```python
from build123d import *

# Parameters (mm, degrees)
L_BRACKET_BODY_DEPTH           = 100
MOUNTING_HOLES_SKETCH_R        = 7
MOUNTING_HOLES_2X_14_DEPTH     = 100
TRUNNION_SKETCH_R              = 20
TRUNNION_40_DEPTH              = 100
TRUNNION_START                 = 5
TRUNNION_END_BOSS_A_SKETCH_R   = 20
TRUNNION_END_BOSS_A_40X5_DEPTH = 5
TRUNNION_END_BOSS_B_SKETCH_R   = 20
TRUNNION_END_BOSS_B_40X5_DEPTH = 5
TRUNNION_BORE_SKETCH_R         = 10
TRUNNION_BORE_20_DEPTH         = 110


with BuildPart() as part:
    # L Bracket Profile Sketch → L Bracket Body (new body)
    with BuildSketch(Plane.XY):
        Polygon((0, 0), (125, 0), (125, 42.5), (16, 42.5), (16, 85), (0, 85), align=None)
    extrude(amount=-L_BRACKET_BODY_DEPTH)

    # Mounting Holes Sketch → Mounting Holes 2xØ14 (cut)
    with BuildSketch(Plane(origin=(16, 0, 0), x_dir=(0, 0, -1), z_dir=(1, 0, 0))):
        with Locations((18, 68)):
            Circle(MOUNTING_HOLES_SKETCH_R)
        with Locations((82, 68)):
            Circle(MOUNTING_HOLES_SKETCH_R)
    extrude(amount=-MOUNTING_HOLES_2X_14_DEPTH, mode=Mode.SUBTRACT)

    # Trunnion Sketch → Trunnion Ø40 (add)
    with BuildSketch(Plane.XY):
        with Locations((70.5, 42.5)):
            Circle(TRUNNION_SKETCH_R)
    extrude(amount=-TRUNNION_40_DEPTH)

    # Trunnion End Boss A Sketch → Trunnion End Boss A Ø40x5 (add)
    with BuildSketch(Plane.XY.offset(TRUNNION_START)):
        with Locations((70.5, 42.5)):
            Circle(TRUNNION_END_BOSS_A_SKETCH_R)
    extrude(amount=-TRUNNION_END_BOSS_A_40X5_DEPTH)

    # Trunnion End Boss B Sketch → Trunnion End Boss B Ø40x5 (add)
    with BuildSketch(Plane(origin=(0, 0, -100), x_dir=(-1, 0, 0), z_dir=(0, 0, -1))):
        with Locations(Location((-70.5, 42.5, 0), (0, 0, 180))):
            Circle(TRUNNION_END_BOSS_B_SKETCH_R)
    extrude(amount=TRUNNION_END_BOSS_B_40X5_DEPTH)

    # Trunnion Bore Sketch → Trunnion Bore Ø20 (cut)
    with BuildSketch(Plane(origin=(0, 0, -105), x_dir=(-1, 0, 0), z_dir=(0, 0, -1))):
        with Locations((-70.5, 42.5)):
            Circle(TRUNNION_BORE_SKETCH_R)
    extrude(amount=-TRUNNION_BORE_20_DEPTH, mode=Mode.SUBTRACT)


solid = part.part
```
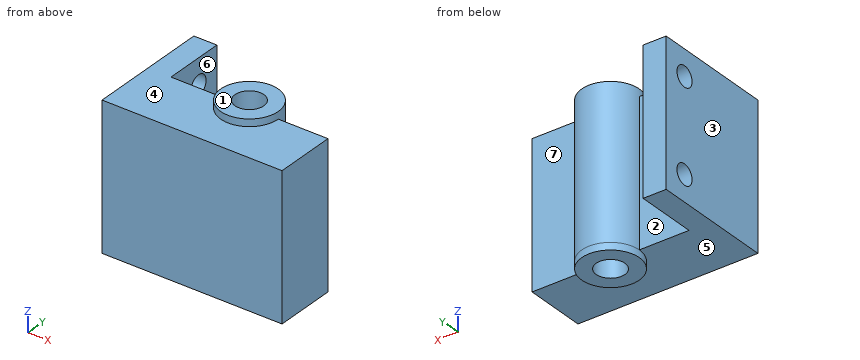
Geometry: final body of the model. Coordinates: model frame, mm. Face numbers are marked on the shaded views. A direction names the side the tool comes from. Round coordinates to 2 decimals unless told otherwise and drop trailing zeros. Order: outer loops, then holes, each group sorted by start corner. A loop starts at its lowest first (then second) coordinate and runs counter-clockwise, first axis right, second up. Notation, with made-up numbers: (76, -15) -> (123, -15) arc R31 cw to (123, 12) -> close; hole circle Ø9 at (10.5, -16). An arc over 180 degrees is marked (long way). Use one line per item in the form item = value.
(1) Section C-C on x = 70.5. Return loops of the section in (y, z).
Results list:
outline = (0, -100) -> (22.5, -100) -> (22.5, -105) -> (32.5, -105) -> (32.5, 5) -> (22.5, 5) -> (22.5, 0) -> (0, 0) -> close; (52.5, -105) -> (62.5, -105) -> (62.5, 5) -> (52.5, 5) -> close
(2) First-contact query: pin 1 Ø8 at (x, z) = (57, -52.5) entering from +Y; pin 2 Ø6 at (x, y) = (74.5, 45) entering from +Z; pin 3 Ø16 at (y, z) = (68, -18) entering from +X; pin 4 Ø3 at (x, z) = (87, -55.5) entering from +Y. Flat tips, straight axial feed; report the tip coordinate or a pass-through.
Results list:
pin_1 = 60.1
pin_2 = through
pin_3 = 80.18
pin_4 = 55.73
(3) Ray query, probe 1 along Y at (x, z) = (3.5, -18); probe 2 along X at (y, z) = (44.5, -1.5); probe 3 along Z at (x, y) = (68.5, 17). Return the intervals inside material, ascending. Write a range as [from, to].
Results list:
probe_1 = [0, 61], [75, 85]
probe_2 = [0, 16], [50.6, 60.7], [80.3, 90.4]
probe_3 = [-100, 0]
(4) Section D-D on z = -7. Return loops of the section in (x, y).
Results list:
outline = (0, 0) -> (125, 0) -> (125, 42.5) -> (90.5, 42.5) arc R20 ccw to (50.5, 42.5) -> (16, 42.5) -> (16, 85) -> (0, 85) -> close; hole circle Ø20 at (70.5, 42.5)
(5) Draft query along X for the marked faces 1, 2 and 3. Return one class per face: pulls with the +X half, pulls with the -X half, needs draft (parallel to the pull), parting line crosses it, or undercut.
Results list:
face_1 = needs draft
face_2 = undercut
face_3 = pulls with the -X half
(6) Access query for the marked faces 4, 5, 6 and 7. Directions: +Z, -Z, +X, -X, +Y, -Y. A direction counts if a zero-diameter tool reaches every point of the face in a straight line with its end or side. Return the directions, or none.
Results list:
face_4 = +Z, -Y
face_5 = -Z, -Y
face_6 = +Z, -Z, +Y
face_7 = +Z, -Z, +X, +Y
(7) Section A-A on z = -82. Return loops of the section in (x, y), and give its area (3 significant figures).
Results list:
outline = (0, 0) -> (125, 0) -> (125, 42.5) -> (90.5, 42.5) arc R20 ccw to (50.5, 42.5) -> (16, 42.5) -> (16, 61) -> (0, 61) -> close; (0, 75) -> (16, 75) -> (16, 85) -> (0, 85) -> close; hole circle Ø20 at (70.5, 42.5)
area = 6,080 mm^2
(8) Section B-B on y = 68. Return loops of the section in (x, z).
Results list:
outline = (0, -100) -> (16, -100) -> (16, -89) -> (0, -89) -> close; (0, -75) -> (16, -75) -> (16, -25) -> (0, -25) -> close; (0, -11) -> (16, -11) -> (16, 0) -> (0, 0) -> close
